```python
from build123d import *

# Parameters (mm, degrees)
M24X2_0_TAPPED_HOLE1_D = 22
SKETCH2_R              = 12.5
CUT_EXTRUDE1_DEPTH     = 1138.348231634
SKETCH4_R              = 37.5
CUT_EXTRUDE2_DEPTH     = 1190.746191421


with BuildPart() as part:
    # Sketch1 → Revolve1 (revolve)
    with BuildSketch(Plane.XY, mode=Mode.PRIVATE) as revolve1_sk:
        with BuildLine():
            Line((0, 0), (0, 185))
            Line((0, 185), (5, 190))
            Line((5, 190), (47, 190))
            Line((47, 190), (47.8, 189.2))
            Line((47.8, 189.2), (53.8, 189.2))
            ThreePointArc((53.8, 189.2), (55.214213562, 189.785786438), (55.8, 191.2))
            Line((55.8, 191.2), (55.8, 197.2))
            Line((55.8, 197.2), (55, 198))
            Line((55, 198), (55, 248))
            Line((55, 248), (57, 250))
            Line((57, 250), (103, 250))
            Line((103, 250), (105, 248))
            Line((105, 248), (105, 130.475))
            ThreePointArc((105, 130.475), (108.807611845, 121.282611845), (118, 117.475))
            Line((118, 117.475), (150, 117.475))
            Line((150, 117.475), (171.607333824, 105))
            Line((171.607333824, 105), (241.215390309, 105))
            Line((241.215390309, 105), (262, 117))
            Line((262, 117), (282, 117))
            Line((282, 117), (282, 113))
            ThreePointArc((282, 113), (282.878679656, 110.878679656), (285, 110))
            Line((285, 110), (392, 110))
            Line((392, 110), (400.660254038, 105))
            Line((400.660254038, 105), (622, 105))
            Line((622, 105), (631.330127019, 102.5))
            Line((631.330127019, 102.5), (1136, 102.5))
            Line((1136, 102.5), (1136, 0))
            Line((1136, 0), (0, 0))
        make_face()
    revolve(revolve1_sk.sketch.rotate(Axis((0, 0, 0), (1, 0, 0)), 90), axis=Axis((0, 0, 0), (1, 0, 0)))

    # M24x2.0 Tapped Hole1 (through all)
    with Locations(Plane(origin=(55, 220, 0), x_dir=(0, 0, -1), z_dir=(-1, 0, 0))):
        with Locations((0, 0), (-190.525588833, 110), (190.525588833, 110), (190.525588833, 330), (0, 440), (-190.525588833, 330), (-155.563491861, 64.436508139), (155.563491861, 375.563491861)):
            Hole(M24X2_0_TAPPED_HOLE1_D / 2)

    # Sketch2 → Cut-Extrude1 (cut, through all)
    with BuildSketch(Plane.ZY.offset(-55)):
        with Locations((-110, 190.525588833)):
            Circle(SKETCH2_R)
        with Locations((110, 190.525588833)):
            Circle(SKETCH2_R)
        with Locations((220, 0)):
            Circle(SKETCH2_R)
        with Locations((110, -190.525588833)):
            Circle(SKETCH2_R)
        with Locations((-110, -190.525588833)):
            Circle(SKETCH2_R)
        with Locations((-220, 0)):
            Circle(SKETCH2_R)
    extrude(amount=-CUT_EXTRUDE1_DEPTH, mode=Mode.SUBTRACT)

    # Sketch4 → Cut-Extrude2 (cut, through all)
    with BuildSketch(Plane(origin=(1136, 0, 0), x_dir=(0, 0, -1), z_dir=(1, 0, 0))):
        Circle(SKETCH4_R)
    extrude(amount=-CUT_EXTRUDE2_DEPTH, mode=Mode.SUBTRACT)


solid = part.part
```
Here's how the part is built. I have some questions about the finished solid (model axes, mm). A direction names the side the tool comes from. Round coordinates to 2 decimals unless told otherwise and drop trailing zeros. Order: outer loops, then holes, each group sorted by start corner. A loop starts at its lowest first (then second) coordinate and runs counter-clockwise, first axis right, second up. Notation, with made-up numbers: (88.5, 56) -> (126.5, 56) arc R22 cw to (126.5, 95) -> close; hole circle Ø11 at (33.25, 68). An arc over 180 degrees is marked (long way). Use a Markdown table: item, result. Add a question column.
(1) Suppose I cut it at B-B, the plane x = 307. Please give me the cut outline in (y, z), and give its area (3 significant figures).
(2) For pin 1 Ø22.5 at (y, z) = (190.53, 110) entering from -X; pin 2 Ø8 at (x, z) = (838, -45.5) entering from +Y; pin 3 Ø1.5 at (x, y) = (268.5, 107) entering from +Z; pin 4 Ø4 at (y, z) = (-196.5, -69.5) entering from +X, each with a flat end and sliding along its axis, tell me the tip position at first contact or that it passes through.
(3) For faces 1 (the face through (80.35, -230.906, -1.432)), 2 (the face through (887.198, 100.063, -22.22)), 3 (the face through (55, -185, 75)), which set-ups out of +Z, -Z, +X, -X, +Y, -Y let a thin tool reach every point of the face, with its end or its side?
(4) I need wall thicknesses on line 1 along Y through (x, z) = (646, 0); line 2 along Z through (x, y) = (65, -110); line 3 along X through (y, z) = (91.5, -224.5). Which ranges of each line are inside material? Lowest first, please.
(5) If we mould it in two halves opening along X, with no side actions, what happens to faces 4 (the face through (242.52, -4.65, -105.65)), 5 (the face through (630.877, -30.825, 97.883)), 6 (the face through (79.6, -201.6, -104.2))? For each: released by +X, released by -X, zero draft, split by the parting line, or undercut.
(6) Suppose I cut it at A-A, the plane z = 0. Count the separate pieces of the cut face and the enclosed holes in it, and give its area (3 significant figures).
Verdict:
| question | item | result |
|---|---|---|
| 1 | outline | circle Ø220 at (0, 0); hole circle Ø75 at (0, 0) |
| 1 | area | 33,600 mm2 |
| 2 | pin 1 | through |
| 2 | pin 2 | y = 93.72 |
| 2 | pin 3 | z = 48.99 |
| 2 | pin 4 | x = 105 |
| 3 | face 1 | +X, -X |
| 3 | face 2 | +X |
| 3 | face 3 | -X |
| 4 | line 1 | -102.5 to -37.5, 37.5 to 102.5 |
| 4 | line 2 | -224.5 to -201.53, -179.53 to 179.53, 201.53 to 224.5 |
| 4 | line 3 | 55 to 105 |
| 5 | face 4 | undercut |
| 5 | face 5 | released by +X |
| 5 | face 6 | zero draft |
| 6 | separate pieces | 4 |
| 6 | enclosed holes | 0 |
| 6 | area | 176,000 mm2 |
